Geometry: final body of the model. Coordinates: model frame, mm. A direction names the side the tool comes from. Round coordinates to 2 decimals unless told otherwise and drop trailing zeros. Write each loop counter-clockwise with the first axis right and the second up, starting at its lowest first coordinate (ties: lowest second). Pieces come first, ordered by that corner, then holes. Notation, with made-up numbers: (76, -34) - (132, -34) arc R7 ccw to (132, -22) - close; hole circle Ø8 at (-26, 11.5). An arc over 180 degrees is marked (long way). Write each question's results on one line, items separated by ' | '.
from build123d import *

# Parameters (mm, degrees)
BASE_PLATE_SKETCH_W              = 70
BASE_PLATE_SKETCH_H              = 25
BASE_PLATE_70X25X5_DEPTH         = 5
TWIN_PILLARS_DEPTH               = 25
CROSS_HOLES_SKETCH_R             = 4
CROSS_HOLES_2X_8_DEPTH           = 35
RELIEF_SLOT_SKETCH_W             = 10
RELIEF_SLOT_SKETCH_H             = 3
UNDERSIDE_RELIEF_SLOT_10X3_DEPTH = 35


with BuildPart() as part:
    # Base Plate Sketch → Base Plate 70x25x5 (new body)
    with BuildSketch(Plane(origin=(0, 0, 0), x_dir=(1, 0, 0), z_dir=(0, 1, 0))):
        with Locations((35, 12.5)):
            Rectangle(BASE_PLATE_SKETCH_W, BASE_PLATE_SKETCH_H)
    extrude(amount=BASE_PLATE_70X25X5_DEPTH)

    # Pillar Profile Sketch → Twin Pillars (add)
    with BuildSketch(Plane.XY):
        Polygon((9, 5), (9, 23), (19, 30), (29, 23), (29, 20), (41, 20), (41, 23), (51, 30), (61, 23), (61, 5), align=None)
    extrude(amount=-TWIN_PILLARS_DEPTH)

    # Cross Holes Sketch → Cross Holes 2xØ8 (cut)
    with BuildSketch(Plane.XY):
        with Locations((51, 15)):
            Circle(CROSS_HOLES_SKETCH_R)
        with Locations((19, 15)):
            Circle(CROSS_HOLES_SKETCH_R)
    extrude(amount=-CROSS_HOLES_2X_8_DEPTH, mode=Mode.SUBTRACT)

    # Relief Slot Sketch → Underside Relief Slot 10x3 (cut)
    with BuildSketch(Plane.XY):
        with Locations((35.488696345, 1.5)):
            Rectangle(RELIEF_SLOT_SKETCH_W, RELIEF_SLOT_SKETCH_H)
    extrude(amount=-UNDERSIDE_RELIEF_SLOT_10X3_DEPTH, mode=Mode.SUBTRACT)


solid = part.part
Q1. Access query for faces 1 (the flat face through (40.489, 1, -12)), 2 (the flat face through (4, 5, -13)), 3 (the flat face through (35, 20, -12)). Directions: +Z, -Z, +X, -X, +Y, -Y. A direction counts if a zero-diameter tool reaches every point of the face in a straight line with its end or side. Return the directions, or none.
Answer block:
face 1: +Z, -Z, -Y | face 2: +Z, -Z, -X, +Y | face 3: +Z, -Z, +Y
Q2. Section query D-D, the plane x = 17. Return loops of the section in (y, z), plus the area to 3 significant figures.
Answer block:
outline: (0, -25) - (11.54, -25) - (11.54, 0) - (0, 0) - close; (18.46, -25) - (28.6, -25) - (28.6, 0) - (18.46, 0) - close | area: 542 mm2
Q3. Mould query, pull axis X, two halves, no side actions, for faces 4 (the flat face through (70, 2, -12)), 5 (the flat face through (30.489, 1, -12)), 6 (the flat face through (9, 14, -12)), 7 (the flat face through (35, 11, 0)). Classes: pulls with the +X half, pulls with the -X half, needs draft (parallel to the pull), parting line crosses it, or undercut.
Answer block:
face 4: pulls with the +X half | face 5: undercut | face 6: pulls with the -X half | face 7: needs draft
Q4. Section query C-C, the plane z = -22.5. Return loops of the section in (x, y), plus the area to 3 significant figures.
Answer block:
outline: (0, 0) - (30.49, 0) - (30.49, 3) - (40.49, 3) - (40.49, 0) - (70, 0) - (70, 5) - (61, 5) - (61, 23) - (51, 30) - (41, 23) - (41, 20) - (29, 20) - (29, 23) - (19, 30) - (9, 23) - (9, 5) - (0, 5) - close; hole circle Ø8 at (19, 15); hole circle Ø8 at (51, 15) | area: 1,260 mm2
Q5. Section query A-A, the plane y = 15. Return loops of the section in (x, z).
Answer block:
outline: (9, -25) - (15, -25) - (15, 0) - (9, 0) - close; (23, -25) - (47, -25) - (47, 0) - (23, 0) - close; (55, -25) - (61, -25) - (61, 0) - (55, 0) - close
Q6. Pin query (flat end, axial travel): pin 1 (3 mm diameter, centred on x = 35.5, z = -11.5, fed in from +Y); pin 2 (2 mm diameter, centred on x = 9, z = -11, fed in from +Y); pin 3 (5 mm diameter, centred on x = 36, z = -13, fed in from -Y); pin 4 (6.5 mm diameter, centred on x = 19, y = 15, fed in from +Z). Return the tip coordinate at first contact, or that it passes through.
Answer block:
pin 1: y = 20 | pin 2: y = 23.7 | pin 3: y = 3 | pin 4: through
Q7. Section query B-B, the plane y = 22. Return loops of the section in (x, z).
Answer block:
outline: (9, -25) - (29, -25) - (29, 0) - (9, 0) - close; (41, -25) - (61, -25) - (61, 0) - (41, 0) - close
Q8. Ray query, line 1 along Y through (x, z) = (19, -18.5); line 2 along X through (y, z) = (14, -4.5); line 3 along X through (y, z) = (8.5, -2.75). Return the intervals inside material, ascending.
Answer block:
line 1: 0 to 11, 19 to 30 | line 2: 9 to 15.13, 22.87 to 47.13, 54.87 to 61 | line 3: 9 to 61
